The listing builds one solid part. Answer for the finished solid, in the listing's coordinates (mm). Face numbers are marked on the shaded views. A direction names the side the tool comes from. Give positions to 0.01 mm unless a question says otherwise; leave off trailing zeros. Loops run counter-clockwise (first coordinate to the right, second up) from the corner with the lowest first, then second, coordinate; pieces in that order, holes last. Notation, with made-up numbers: M 84,-30 L 116,-30 A22 cw 116,-8 Z; hole C 67,-3 d1. An arc over 180 degrees is marked long. One line per item, written item: value. Start each with the question number.
Q1. Consider L1, parallel to Y at x = 23, z = -1.85; L2, parallel to X at y = 23, z = -9; L3, parallel to Y at x = 54, z = -1.5. Determine where each line is inside the solid, lowest interval first.
Q2. A cutting plane is placed at B-B, the plane x = 23. Determine the outline of the cut face in (y, z), and give its area (3 significant figures).
Q3. The mould has two halves that part along X. Classify the marked faces 1, 2 and 3: +X half, -X half, draft (parallel to the pull), parting line (faces both ways), or undercut.
Q4. Flat-ended cylindrical pins translate along their axes: pin 1 (3 mm diameter, centred on x = 53, y = 42.5, fed in from -Z); pin 2 (4 mm diameter, centred on x = 23, y = 7.5, fed in from -Z); pin 3 (2 mm diameter, centred on x = 23, y = 42.5, fed in from -Z); pin 4 (2.5 mm diameter, centred on y = 27, z = -9.5, fed in from +X). Find the tip coordinate at first contact, or state that the pin passes through.
Q5. A cutting plane is placed at D-D, the plane y = 31. Determine the outline of the cut face in (x, z).
Q6. A cutting plane is placed at C-C, the plane z = -9. Determine the outline of the cut face in (x, y), and give its area (3 significant figures).
Q7. A cutting plane is placed at A-A, the plane y = 42.5. Determine the outline of the cut face in (x, z), and give its area (3 significant figures).
Q8. For the marked faces 4 and 5, determine the directions among +Z, -Z, +X, -X, +Y, -Y from which every point of the face is accessible in a straight line to the end or side of a thin tool.
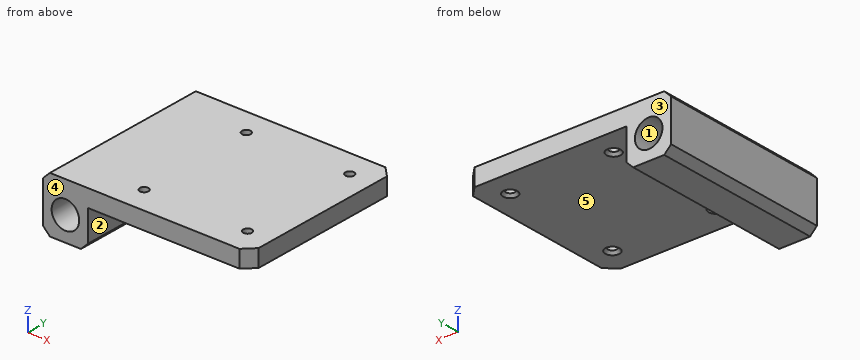
from build123d import *

# Parameters (mm, degrees)
BOSS_EXTRUDE1_DEPTH   = 50
SKETCH2_R             = 0.75
CUT_EXTRUDE1_DEPTH    = 10
SKETCH3_R             = 4
CUT_EXTRUDE2_DEPTH    = 60
CHAMFER1_SIZE         = 2
LPATTERN1_COUNT       = 2
LPATTERN1_PITCH       = 30
CHAMFER2_SIZE         = 3
M3_TAPPED_HOLE1_D     = 2.5
M3_TAPPED_HOLE1_DEPTH = 7.5
M3_TAPPED_HOLE1_TIP   = 0.751075774
CHAMFER3_SIZE         = 0.8


with BuildPart() as part:
    # Sketch1 → Boss-Extrude1 (new body)
    with BuildSketch(Plane(origin=(0, 0, 0), x_dir=(1, 0, 0), z_dir=(0, 1, 0))):
        Polygon((0, 0), (60, 0), (60, 5), (13, 5), (13, 16), (0, 16), align=None)
    extrude(amount=BOSS_EXTRUDE1_DEPTH)

    # Sketch2 → Cut-Extrude1 (cut)
    with BuildSketch(Plane.XY):
        with Locations((53, 42.5)):
            Circle(SKETCH2_R)
        with Locations((53, 7.5)):
            Circle(SKETCH2_R)
    cut_extrude1 = extrude(amount=-CUT_EXTRUDE1_DEPTH, mode=Mode.SUBTRACT)

    # Sketch3 → Cut-Extrude2 (cut)
    with BuildSketch(Plane(origin=(0, 50, 0), x_dir=(1, 0, 0), z_dir=(0, 1, 0))):
        with Locations(Location((6.5, 9, 0), (0, 0, 270))):
            Circle(SKETCH3_R)
    extrude(amount=-CUT_EXTRUDE2_DEPTH, mode=Mode.SUBTRACT)

    # Chamfer1
    chamfer1_edges = [part.edges().sort_by_distance(p)[0] for p in [
        (0, 25, -16),
        (13, 25, -16),
        (0, 25, 0),
    ]]
    chamfer(chamfer1_edges, length=CHAMFER1_SIZE)

    # LPattern1: Cut-Extrude1 ×2
    with Locations(*[(-i * LPATTERN1_PITCH, 0, 0) for i in range(1, LPATTERN1_COUNT)]):
        add(cut_extrude1, mode=Mode.SUBTRACT)

    # Chamfer2
    chamfer2_edges = [part.edges().sort_by_distance(p)[0] for p in [
        (60, 50, -2.5),
        (60, 0, -2.5),
    ]]
    chamfer(chamfer2_edges, length=CHAMFER2_SIZE)

    # M3 Tapped Hole1
    with Locations(Plane(origin=(23, 42.5, 0), x_dir=(1, 0, 0), z_dir=(0, 0, 1))):
        with Locations((0, 0), (30, 0), (30, -35), (0, -35)):
            Hole(M3_TAPPED_HOLE1_D / 2, depth=M3_TAPPED_HOLE1_DEPTH)
            with Locations((0, 0, -(M3_TAPPED_HOLE1_DEPTH + M3_TAPPED_HOLE1_TIP / 2))):  # 118° drill point
                Cone(0, M3_TAPPED_HOLE1_D / 2, M3_TAPPED_HOLE1_TIP, mode=Mode.SUBTRACT)

    # Chamfer3
    chamfer3_edges = [part.edges().sort_by_distance(p)[0] for p in [
        (24.25, 7.5, -5),
        (54.25, 7.5, -5),
        (54.25, 42.5, -5),
        (24.25, 42.5, -5),
    ]]
    chamfer(chamfer3_edges, length=CHAMFER3_SIZE)


solid = part.part
Answer block:
1. L1: 0 to 6.25, 8.75 to 41.25, 43.75 to 50
1. L2: 0 to 2.5, 10.5 to 13
1. L3: 0 to 6.75, 8.25 to 41.75, 43.25 to 50
2. outline: M 0,-5 L 5.45,-5 L 6.25,-4.2 L 6.25,0 L 0,0 Z; M 8.75,-4.2 L 9.55,-5 L 40.45,-5 L 41.25,-4.2 L 41.25,0 L 8.75,0 Z; M 43.75,-4.2 L 44.55,-5 L 50,-5 L 50,0 L 43.75,0 Z
2. area: 224 mm^2
3. face 1: undercut
3. face 2: +X half
3. face 3: draft
4. pin 1: z = -4.45
4. pin 2: z = -4.95
4. pin 3: through
4. pin 4: x = 13
5. outline: M 0,-14 L 2,-16 L 11,-16 L 13,-14 L 13,-5 L 60,-5 L 60,0 L 2,0 L 0,-2 Z; hole C 6.5,-9 d8
6. outline: M 0,0 L 2.5,0 L 2.5,50 L 0,50 Z; M 10.5,0 L 13,0 L 13,50 L 10.5,50 Z
6. area: 250 mm^2
7. outline: M 0,-14 L 2,-16 L 11,-16 L 13,-14 L 13,-5 L 20.95,-5 L 21.75,-4.2 L 21.75,0 L 2,0 L 0,-2 Z; M 24.25,-4.2 L 25.05,-5 L 50.95,-5 L 51.75,-4.2 L 51.75,0 L 24.25,0 Z; M 54.25,-4.2 L 55.05,-5 L 60,-5 L 60,0 L 54.25,0 Z; hole C 6.5,-9 d8
7. area: 360 mm^2
8. face 4: +Z, -Z, +X, -X, -Y
8. face 5: -Z, +X, +Y, -Y
